```python
from build123d import *

# Parameters (mm, degrees)
SKETCH1_R                                    = 50
SKETCH1_R_2                                  = 12.75
BOSS_EXTRUDE1_DEPTH                          = 3
CSK_FOR_M4_HEX_SOCKET_COUNTERSUNK_CA_2_COUNT = 2
CSK_FOR_M4_HEX_SOCKET_COUNTERSUNK_CA_2_PITCH = 26.811555509
CSK_FOR_M4_HEX_SOCKET_COUNTERSUNK_CA_3_COUNT = 2
CSK_FOR_M4_HEX_SOCKET_COUNTERSUNK_CA_3_PITCH = 14.791639161


with BuildPart() as part:
    # Sketch1 → Boss-Extrude1 (new body)
    with BuildSketch(Plane.XY):
        Circle(SKETCH1_R)
        Circle(SKETCH1_R_2, mode=Mode.SUBTRACT)
    extrude(amount=BOSS_EXTRUDE1_DEPTH)

    # Sketch2 → CSK for M4 Hex Socket Countersunk Cap Screw1 (revolve, cut)
    with BuildSketch(Plane(origin=(5.985352508, 16.444620864, 0), x_dir=(0, 1, 0), z_dir=(1, 0, 0))):
        Polygon((0, 0), (0, 3), (2.4, 3), (2.4, 2.08), (4.48, 0), align=None)
    csk_for_m4_hex_socket_countersunk_cap_sc = revolve(axis=Axis((5.985352508, 16.444620864, -6.35), (0, 0, 1)), mode=Mode.SUBTRACT)

    # CSK for M4 Hex Socket Countersunk Ca 2: CSK for M4 Hex Socket Countersunk Cap Screw1 ×2
    with Locations(*[Vector(0.3420201433256698, -0.9396926207859081, 0) * (i * CSK_FOR_M4_HEX_SOCKET_COUNTERSUNK_CA_2_PITCH) for i in range(1, CSK_FOR_M4_HEX_SOCKET_COUNTERSUNK_CA_2_COUNT)]):
        add(csk_for_m4_hex_socket_countersunk_cap_sc, mode=Mode.SUBTRACT)

    # CSK for M4 Hex Socket Countersunk Ca 3: CSK for M4 Hex Socket Countersunk Cap Screw1 ×2
    with Locations(*[Vector(0.7071067811865491, -0.707106781186546, 0) * (i * CSK_FOR_M4_HEX_SOCKET_COUNTERSUNK_CA_3_PITCH) for i in range(1, CSK_FOR_M4_HEX_SOCKET_COUNTERSUNK_CA_3_COUNT)]):
        add(csk_for_m4_hex_socket_countersunk_cap_sc, mode=Mode.SUBTRACT)


solid = part.part
```
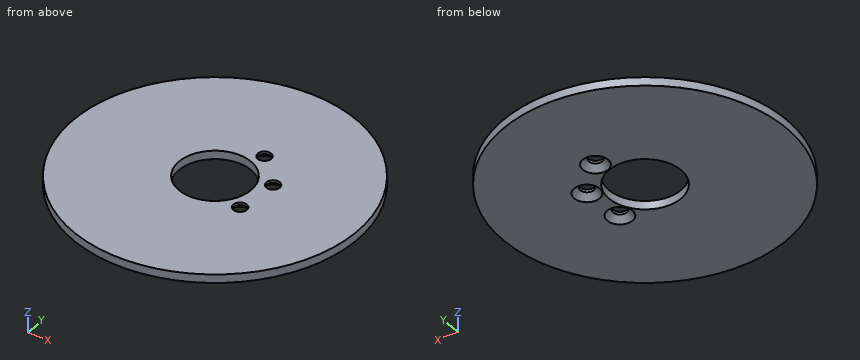
Build history of the part. All positions in model axes, mm. Coordinates: 2 decimals unless noted, no trailing zeros. Order: outer loops, then holes, each group sorted by start corner. A loop starts at its lowest first (then second) coordinate and runs counter-clockwise, first axis right, second up. Notation, with made-up numbers: (32, 86) -> (46, 86) arc R30 cw to (46, 122) -> close; hole circle Ø5 at (45, 86.25). An arc over 180 degrees is marked (long way). Answer in a Markdown table with one row per item. Add a question column.
Q1. Drop flat-ended pins along their axis: pin 1 (4.5 mm diameter, centred on x = 15.16, y = -8.75, fed in from +Z); pin 2 (1.5 mm diameter, centred on y = 13, z = 1.5, fed in from -X). Give the stop position or say it passes through.
Q2. Wall check: line 1 along Y through (x, z) = (18.5, 0.6); line 2 along X through (y, z) = (-8.75, 2.6); line 3 along Y through (x, z) = (0, 1.85). Give the ranges that are in metal, low to high. Write a range as [from, to].
Q3. Band-saw the part on C-C, the plane z = 1.1. List the corners of the cut face in (x, y).
Q4. Band-saw the part on A-A, the plane x = 0. List the corners of the cut face in (y, z).
Q5. Band-saw the part on D-D, the plane x = 25. List the corners of the cut face in (y, z).
Answers follow:
| question | item | result |
|---|---|---|
| 1 | pin 1 | through |
| 1 | pin 2 | x = -48.48 |
| 2 | line 1 | [-46.45, -10.72], [-6.78, 2.69], [9.28, 46.45] |
| 2 | line 2 | [-49.23, -9.27], [9.27, 12.76], [17.56, 49.23] |
| 2 | line 3 | [-50, -12.75], [12.75, 50] |
| 3 | outline | circle Ø100 at (0, 0); hole circle Ø25.5 at (0, 0); hole circle Ø6.76 at (5.99, 16.44); hole circle Ø6.76 at (15.16, -8.75); hole circle Ø6.76 at (16.44, 5.99) |
| 4 | outline | (-50, 0) -> (-12.75, 0) -> (-12.75, 3) -> (-50, 3) -> close; (12.75, 0) -> (50, 0) -> (50, 3) -> (12.75, 3) -> close |
| 5 | outline | (-43.3, 0) -> (43.3, 0) -> (43.3, 3) -> (-43.3, 3) -> close |
